Job drawing, mm, ordinate dimensions from the low corner. One solid piece. A direction names the side the tool comes from. Give positions to 0.01 mm unless a question says otherwise; leave off trailing zeros. Order: outer loops, then holes, each group sorted by start corner. A loop starts at its lowest first (then second) coordinate and runs counter-clockwise, first axis right, second up. Notation, with made-up numbers: (-16, 57.5) - (40, 57.5) arc R9 ccw to (40, 72.5) - close; hole circle Ø10 at (20.5, 74.25). An arc over 180 degrees is marked (long way). Write each question's results on one line, items separated by ' | '. Start each with the question number.
1) Two-plate mould, pull along Y, no slides. Class the marked faces 1, 2, 3 and 4: +Y half, -Y half, draft (parallel to the pull), parting line (faces both ways), or undercut.
2) Drop flat-ended pins along their axis: pin 1 Ø10 at (x, y) = (37.5, 49) entering from +Z; pin 2 Ø10 at (x, z) = (20.5, 118.5) entering from +Y; pin 3 Ø10 at (x, z) = (40.5, 103) entering from -Y. Give the stop position or say it passes through.
3) Cut at D-D on x = 62.5. List the corners of the cut face in (y, z).
4) Drill centre lines: line 1 along Y through (x, z) = (36.5, 30); line 2 along X through (y, z) = (39, 20); line 3 along Y through (x, z) = (88.5, 116). Where is each one in solid material? Low to high. Write a range as from..to.
5) Cut at B-B on y = 56. List the corners of the cut face in (x, z), plus the area to 3 significant figures.
6) Cut at A-A on x = 48.5. List the corners of the cut face in (y, z).
7) Tool access for the marked faces 5, 6 and 7: list every direction of +Z, -Z, +X, -X, +Y, -Y with a clear straight run to the whole face (end or side of a thin tool).
8) Cut at C-C on z = 120. List the corners of the cut face in (x, y) (1 decimal).
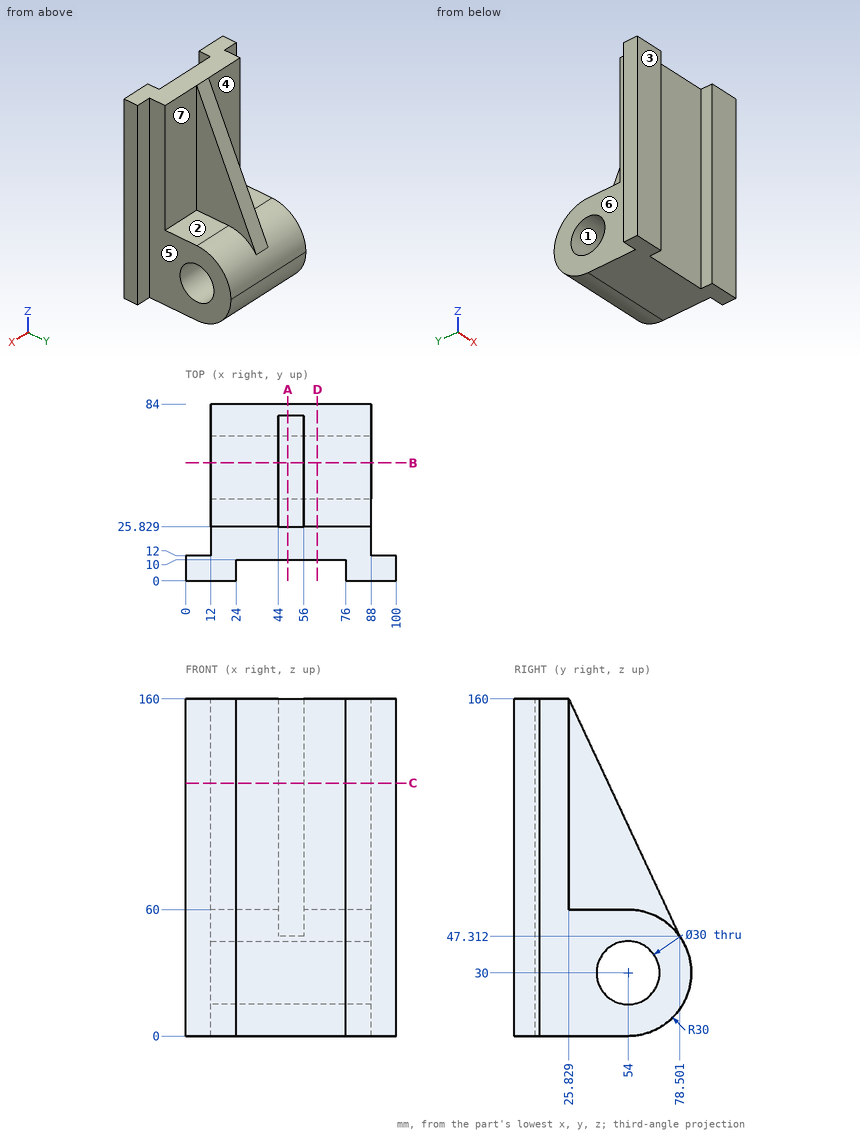
Results:
1) face 1: undercut | face 2: draft | face 3: -Y half | face 4: +Y half
2) pin 1: z = 60 | pin 2: y = 25.83 | pin 3: y = 10
3) outline: (10, 0) - (54, 0) arc R30 ccw to (54, 60) - (25.83, 60) - (25.83, 160) - (10, 160) - close; hole circle Ø30 at (54, 30)
4) line 1: 10..39, 69..84 | line 2: 12..88 | line 3: 0..12
5) outline: (12, 0.07) - (88, 0.07) - (88, 15.13) - (12, 15.13) - close; (12, 44.87) - (88, 44.87) - (88, 59.93) - (56, 59.93) - (56, 95.45) - (44, 95.45) - (44, 59.93) - (12, 59.93) - close | area: 2,720 mm^2
6) outline: (10, 0) - (54, 0) arc R30 ccw to (78.5, 47.31) - (25.83, 160) - (10, 160) - close; hole circle Ø30 at (54, 30)
7) face 5: +Z, -Z, +X, +Y | face 6: +Z, -Z, -X, +Y | face 7: +Z, +X, +Y
8) outline: (0, 0) - (24, 0) - (24, 10) - (76, 10) - (76, 0) - (100, 0) - (100, 12) - (88, 12) - (88, 25.8) - (56, 25.8) - (56, 44.5) - (44, 44.5) - (44, 25.8) - (12, 25.8) - (12, 12) - (0, 12) - close
